from build123d import *

# Parameters (mm, degrees)
EXTRUDE_1_DEPTH              = 6
SKETCH_2_W                   = 2
SKETCH_2_H                   = 8
CUT_EXTRUDE_1_DEPTH          = 20
FILLET_1_R                   = 2
HOLE_WIZARD_M3_1_D           = 3.4
HOLE_WIZARD_M3_1_CBORE_D     = 6
HOLE_WIZARD_M3_1_CBORE_DEPTH = 3.4


with BuildPart() as part:
    # 草图1 → 凸台-拉伸1 (new, symmetric)
    with BuildSketch(Plane.XY):
        Polygon((0, 0), (0, -20.071067812), (9.928932188, -30), (17.5, -30), (17.5, -25), (12, -25), (7, -20), (7, 0), align=None)
    extrude(amount=EXTRUDE_1_DEPTH, both=True)

    # 草图2 → 切除-拉伸1 (cut)
    with BuildSketch(Plane(origin=(0, 0, 0), x_dir=(1, 0, 0), z_dir=(0, 1, 0))):
        with Locations((6, 0)):
            Rectangle(SKETCH_2_W, SKETCH_2_H)
    extrude(amount=-CUT_EXTRUDE_1_DEPTH, mode=Mode.SUBTRACT)

    # 圆角1
    fillet_1_edges = [part.edges().sort_by_distance(p)[0] for p in [
        (6, -20, 4),
        (6, -20, -4),
    ]]
    fillet(fillet_1_edges, radius=FILLET_1_R)

    # M3 六角圆柱头螺钉的柱形沉头孔1 (through all)
    with Locations(Plane.ZY):
        with Locations((0, -4.7), (0, -11.7)):
            CounterBoreHole(HOLE_WIZARD_M3_1_D / 2, HOLE_WIZARD_M3_1_CBORE_D / 2, HOLE_WIZARD_M3_1_CBORE_DEPTH)


solid = part.part
The model under review builds one solid part; all positions refer to its coordinate system, in mm. A direction names the side the tool comes from. Give positions to 0.01 mm unless a question says otherwise; leave off trailing zeros. Loops run counter-clockwise (first coordinate to the right, second up) from the corner with the lowest first, then second, coordinate; pieces in that order, holes last. Notation, with made-up numbers: (17, 87.5) -> (56, 87.5) arc R22 ccw to (56, 124.5) -> close; hole circle Ø6 at (-11, 68). An arc over 180 degrees is marked (long way). Put each result on its own line as item: value. Start each with the question number.
1. We need section C-C on x = 4.5. State the section outline as (y, z) points, then the cut area to 3 significant figures.
2. Mouldability with a two-part tool opening along Y and no side actions: class faces 1 (the face through (7, -10, 5)), 2 (the face through (4, -10, 0)), 3 (the face through (6, -20, 0)), 4 (the face through (3.4, -12, 2)) as released by +Y, released by -Y, zero draft, split by the parting line, or undercut.
3. Wall thickness on probe 1 along Z at (x, y) = (6.25, -4.75); probe 2 along X at (y, z) = (-11.25, 5); probe 3 along X at (y, z) = (-15.75, -0.5): over which ranges is each line inside the solid? List them lowest first.
4. We need section B-B on y = -11.7. State the section outline as (x, z) points, then the cut area to 3 significant figures.
5. Clearance check with flat-ended pins moving along their axes: P1, Ø6, axis at y = -25.5, z = 3, coming from the -X side; P2, Ø0.6, axis at x = 5.5, z = 0, coming from the +Y side; P3, Ø1.8, axis at y = -12, z = 1, coming from the -X side; P4, Ø5, axis at y = -19, z = -1.5, coming from the -X side. State where each tip first meets the part, or that it passes through.
6. We need section A-A on z = 0. State the section outline as (x, y) points.
7. We need section D-D on z = 4.5. State the section outline as (x, y) points, then the cut area to 3 significant figures.
8. For faces 5 (the face through (3.4, -5, 2)), 6 (the face through (6, -9, -4)), 7 (the face through (0, -10, 3)), 8 (the face through (3, 0, 0)), 9 (the face through (7, -10, -5)), list the 3-axis set-ups (+Z, -Z, +X, -X, +Y, -Y) from which the entire face can be reached by the end or side of a thin tool; tool diameter is ignored.
Determined:
1. outline: (-24.57, -6) -> (0, -6) -> (0, 6) -> (-24.57, 6) -> close; hole circle Ø3.4 at (-11.7, 0); hole circle Ø3.4 at (-4.7, 0)
1. area: 277 mm^2
2. face 1: zero draft
2. face 2: undercut
2. face 3: released by +Y
2. face 4: undercut
3. probe 1: -6 to -4, 4 to 6
3. probe 2: 0 to 7
3. probe 3: 0 to 5
4. outline: (0, -6) -> (7, -6) -> (7, -4) -> (5, -4) -> (5, -1.7) -> (3.4, -1.7) -> (3.4, -3) -> (0, -3) -> close; (0, 3) -> (3.4, 3) -> (3.4, 1.7) -> (5, 1.7) -> (5, 4) -> (7, 4) -> (7, 6) -> (0, 6) -> close
4. area: 42.2 mm^2
5. P1: x = 2.43
5. P2: y = -20
5. P3: x = 3.4
5. P4: x = 0
6. outline: (0, -20.07) -> (9.93, -30) -> (17.5, -30) -> (17.5, -25) -> (12, -25) -> (7, -20) -> (5, -20) -> (5, -13.4) -> (3.4, -13.4) -> (3.4, -14.7) -> (0, -14.7) -> close; (0, -8.7) -> (3.4, -8.7) -> (3.4, -10) -> (5, -10) -> (5, -6.4) -> (3.4, -6.4) -> (3.4, -7.7) -> (0, -7.7) -> close; (0, -1.7) -> (3.4, -1.7) -> (3.4, -3) -> (5, -3) -> (5, 0) -> (0, 0) -> close
7. outline: (0, -20.07) -> (9.93, -30) -> (17.5, -30) -> (17.5, -25) -> (12, -25) -> (7, -20) -> (7, 0) -> (0, 0) -> close
7. area: 226 mm^2
8. face 5: -X
8. face 6: +X, +Y
8. face 7: +Z, -Z, -X, +Y, -Y
8. face 8: +Z, -Z, +X, -X, +Y
8. face 9: +Z, -Z, +X, +Y
